Can you work these out from the model? Positions are in its coordinate system, mm. Give positions to 0.01 mm unless a question says otherwise; leave off trailing zeros. Write each loop counter-clockwise with the first axis right and the second up, starting at its lowest first coordinate (ties: lowest second). Pieces come first, ordered by that corner, then holes. Notation, with made-up numbers: (49, 19) - (61, 19) arc R23 ccw to (61, 55) - close; hole circle Ø3 at (7, 15.25). An arc over 180 degrees is marked (long way). Return JSON: item names as keys, results as strings. Group by question number.
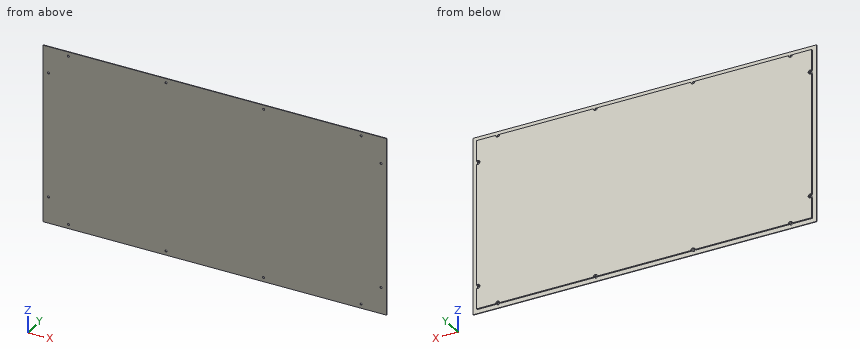
from build123d import *

# Parameters (mm, degrees)
SKETCH1_W           = 493
SKETCH1_H           = 256.3
BOSS_EXTRUDE1_DEPTH = 1.5
SKETCH2_W           = 493
SKETCH2_H           = 256.3
SKETCH2_W_2         = 481
SKETCH2_H_2         = 244.3
CUT_EXTRUDE1_DEPTH  = 2
SKETCH3_R           = 1.5
CUT_EXTRUDE2_DEPTH  = 278.83749297
SKETCH4_R           = 1.5
CUT_EXTRUDE3_DEPTH  = 278.83749297
SKETCH5_R           = 3
CUT_EXTRUDE4_DEPTH  = 2


with BuildPart() as part:
    # Sketch1 → Boss-Extrude1 (new, symmetric)
    with BuildSketch(Plane(origin=(0, 0, 0), x_dir=(1, 0, 0), z_dir=(0, 1, 0))):
        Rectangle(SKETCH1_W, SKETCH1_H)
    extrude(amount=BOSS_EXTRUDE1_DEPTH, both=True)

    # Sketch2 → Cut-Extrude1 (cut)
    with BuildSketch(Plane(origin=(0, 1.5, 0), x_dir=(1, 0, 0), z_dir=(0, 1, 0))):
        Rectangle(SKETCH2_W, SKETCH2_H)
        Rectangle(SKETCH2_W_2, SKETCH2_H_2, mode=Mode.SUBTRACT)
    extrude(amount=-CUT_EXTRUDE1_DEPTH, mode=Mode.SUBTRACT)

    # Sketch3 → Cut-Extrude2 (cut, through all)
    with BuildSketch(Plane(origin=(0, 1.5, 0), x_dir=(1, 0, 0), z_dir=(0, 1, 0))):
        with Locations(Location((-70, 122.15, 0), (0, 0, 270))):
            Circle(SKETCH3_R)
        with Locations(Location((-210, 122.15, 0), (0, 0, 270))):
            Circle(SKETCH3_R)
        with Locations((70, 122.15)):
            Circle(SKETCH3_R)
        with Locations((210, 122.15)):
            Circle(SKETCH3_R)
    cut_extrude2 = extrude(amount=-CUT_EXTRUDE2_DEPTH, mode=Mode.SUBTRACT)

    # Mirror1: Cut-Extrude2 across plane
    add(cut_extrude2.mirror(Plane.XY), mode=Mode.SUBTRACT)

    # Sketch4 → Cut-Extrude3 (cut, through all)
    with BuildSketch(Plane(origin=(0, 1.5, 0), x_dir=(1, 0, 0), z_dir=(0, 1, 0))):
        with Locations(Location((-238.5, 90, 0), (0, 0, 270))):
            Circle(SKETCH4_R)
        with Locations(Location((-238.5, -90, 0), (0, 0, 90))):
            Circle(SKETCH4_R)
    cut_extrude3 = extrude(amount=-CUT_EXTRUDE3_DEPTH, mode=Mode.SUBTRACT)

    # Mirror2: Cut-Extrude3 across plane
    add(cut_extrude3.mirror(Plane(origin=(0, 0, 0), x_dir=(0, 0, 1), z_dir=(1, 0, 0))), mode=Mode.SUBTRACT)

    # Sketch5 → Cut-Extrude4 (cut)
    with BuildSketch(Plane(origin=(0, 1.5, 0), x_dir=(1, 0, 0), z_dir=(0, 1, 0))):
        with Locations((-210, 122.15)):
            Circle(SKETCH5_R)
        with Locations((-70, 122.15)):
            Circle(SKETCH5_R)
        with Locations((70, 122.15)):
            Circle(SKETCH5_R)
        with Locations((210, 122.15)):
            Circle(SKETCH5_R)
        with Locations((238.5, 90)):
            Circle(SKETCH5_R)
        with Locations((238.5, -90)):
            Circle(SKETCH5_R)
        with Locations((210, -122.15)):
            Circle(SKETCH5_R)
        with Locations((70, -122.15)):
            Circle(SKETCH5_R)
        with Locations((-70, -122.15)):
            Circle(SKETCH5_R)
        with Locations((-210, -122.15)):
            Circle(SKETCH5_R)
        with Locations((-238.5, -90)):
            Circle(SKETCH5_R)
        with Locations((-238.5, 90)):
            Circle(SKETCH5_R)
    extrude(amount=-CUT_EXTRUDE4_DEPTH, mode=Mode.SUBTRACT)


solid = part.part
1) I need wall thicknesses on line 1 along Z through (x, y) = (-238.5, -0.75); line 2 along X through (y, z) = (-1.1, -122.15); line 3 along Z through (x, y) = (-210, -1.2). Which ranges of each line are inside material? Lowest first, please.
2) Imagine slicing it at B-B, the plane z = -63.5. Write out the boundary of the cut face in (x, y).
3) Will these pins go through, and if not, where does the flat tip stop? pin 1 Ø3.5 at (x, z) = (238.5, 90) entering from +Y; pin 2 Ø1 at (x, y) = (233.5, 1) entering from -Z; pin 3 Ø2.5 at (x, z) = (-210, -122.15) entering from -Y; pin 4 Ø1.6 at (y, z) = (1, 109.5) entering from -X.
4) Imagine slicing it at A-A, the plane x = 177. Write out the boundary of the cut face in (y, z).
Resolved:
{
 "1": {"line 1": "-128.15 to -91.5, -88.5 to 88.5, 91.5 to 128.15", "line 2": "-246.5 to -211.5, -208.5 to -71.5, -68.5 to 68.5, 71.5 to 208.5, 211.5 to 246.5", "line 3": "-128.15 to -123.65, -120.65 to 120.65, 123.65 to 128.15"},
 "2": {"outline": "(-246.5, -1.5) - (246.5, -1.5) - (246.5, -0.5) - (240.5, -0.5) - (240.5, 1.5) - (-240.5, 1.5) - (-240.5, -0.5) - (-246.5, -0.5) - close"},
 "3": {"pin 1": "y = -0.5", "pin 2": "z = -122.15", "pin 3": "through", "pin 4": "x = -240.5"},
 "4": {"outline": "(-1.5, -128.15) - (-0.5, -128.15) - (-0.5, -122.15) - (1.5, -122.15) - (1.5, 122.15) - (-0.5, 122.15) - (-0.5, 128.15) - (-1.5, 128.15) - close"}
}
